```python
from build123d import *
from OCP.BRepFilletAPI import BRepFilletAPI_MakeChamfer

# Parameters (mm, degrees)
SKETCH_2_R              = 10.5
CUT_EXTRUDE_1_DEPTH     = 133.003787824
HOLE_WIZARD_M24_2_D     = 21
HOLE_WIZARD_M24_2_DEPTH = 63
HOLE_WIZARD_M24_2_TIP   = 6.3090365
CHAMFER_1_SIZE          = 2
CHAMFER_1_SIZE2         = 0.789861687


with BuildPart() as part:
    # 草图1 → 旋转1 (revolve)
    with BuildSketch(Plane.XY, mode=Mode.PRIVATE) as revolve_1_sk:
        Polygon((0, 0), (0, 26.473460386), (20, 30), (105, 30), (125, 26.473460386), (125, 0), align=None)
    revolve(revolve_1_sk.sketch.rotate(Axis((0, 0, 0), (1, 0, 0)), 90), axis=Axis((0, 0, 0), (1, 0, 0)))

    # 草图2 → 切除-拉伸1 (cut, through all)
    with BuildSketch(Plane(origin=(125, 0, 0), x_dir=(0, 0, -1), z_dir=(1, 0, 0))):
        Circle(SKETCH_2_R)
    extrude(amount=-CUT_EXTRUDE_1_DEPTH, mode=Mode.SUBTRACT)

    # M24 螺纹孔2
    with Locations(Plane(origin=(0, 0, 0), x_dir=(0, 0, -1), z_dir=(-1, 0, 0))):
        with Locations((0, 0)):
            Hole(HOLE_WIZARD_M24_2_D / 2, depth=HOLE_WIZARD_M24_2_DEPTH)
            with Locations((0, 0, -(HOLE_WIZARD_M24_2_DEPTH + HOLE_WIZARD_M24_2_TIP / 2))):  # 118° drill point
                Cone(0, HOLE_WIZARD_M24_2_D / 2, HOLE_WIZARD_M24_2_TIP, mode=Mode.SUBTRACT)

    # 倒角1: one chamfer whose edges measure the first distance from different faces: ONE call of the kernel's chamfer builder (chamfer() names one face for all edges)
    chamfer_1_edges_1 = [part.edges().sort_by_distance(p)[0] for p in [
        (0, 0, -26.473460386),
    ]]
    chamfer_1_side_1 = [part.faces().sort_by_distance(p)[0] for p in [
        (10, 0, -28.236730193),
    ]]
    chamfer_1_edges_2 = [part.edges().sort_by_distance(p)[0] for p in [
        (125, 0, -26.473460386),
    ]]
    chamfer_1_side_2 = [part.faces().sort_by_distance(p)[0] for p in [
        (115, 0, -28.236730193),
    ]]
    chamfer_1 = BRepFilletAPI_MakeChamfer(part.part.solid().wrapped)
    for e in chamfer_1_edges_1:
        chamfer_1.Add(CHAMFER_1_SIZE, CHAMFER_1_SIZE2, e.wrapped, chamfer_1_side_1[0].wrapped)  # the first distance lies on this face
    for e in chamfer_1_edges_2:
        chamfer_1.Add(CHAMFER_1_SIZE, CHAMFER_1_SIZE2, e.wrapped, chamfer_1_side_2[0].wrapped)  # the first distance lies on this face
    add(Compound.cast(chamfer_1.Shape()), mode=Mode.REPLACE)


solid = part.part
```
For this review, take the finished solid that the model builds, in its own axes (mm). Round coordinates to 2 decimals unless told otherwise and drop trailing zeros. Write each loop counter-clockwise with the first axis right and the second up, starting at its lowest first coordinate (ties: lowest second). Pieces come first, ordered by that corner, then holes. Notation, with made-up numbers: (2, 9) - (47, 9) arc R12 ccw to (47, 21) - close; hole circle Ø10 at (-34.75, 1.25). An arc over 180 degrees is marked (long way). Put each result on its own line as item: value.
Q1. Mouldability with a two-part tool opening along Y and no side actions: class faces 1 (the face through (0, 0, -11)), 2 (the face through (7.104, 27.067, -6.01)), 3 (the face through (63.4, 3.2, -10)) as released by +Y, released by -Y, zero draft, split by the parting line, or undercut.
Solved:
face 1: zero draft
face 2: split by the parting line
face 3: undercut
Q2. We need section D-D (x = 109.5). Give the boundary of the cut face in (y, z).
Solved:
outline: circle Ø58.41 at (0, 0); hole circle Ø21 at (0, 0)
Q3. We need section C-C (x = 44). Give the boundary of the cut face in (y, z).
Solved:
outline: circle Ø60 at (0, 0); hole circle Ø21 at (0, 0)
Q4. Insertion check: pin 1 Ø2 at (x, y) = (87.5, 6) entering from -Z; pin 2 Ø5 at (x, y) = (87, 9) entering from +Z; pin 3 Ø1 at (x, z) = (58, 1) entering from +Y. Each pin has a flat end and moves straight along its axis. Give the tip position at first contact, or say it passes through.
Solved:
pin 1: stops at z = -29.58
pin 2: stops at z = 29.29
pin 3: stops at y = 30
Q5. Wall thickness on probe 1 along Y at (x, z) = (73, 0); probe 2 along Z at (x, y) = (63, 5.5); probe 3 along Z at (x, y) = (107.5, -9.5): over which ranges is each line inside the solid? List them lowest first.
Solved:
probe 1: y = -30 to -10.5, 10.5 to 30
probe 2: z = -29.49 to -8.94, 8.94 to 29.49
probe 3: z = -27.99 to -4.47, 4.47 to 27.99
Q6. We need section A-A (z = 0). Give the boundary of the cut face in (x, y), and give its area (3 significant figures).
Solved:
outline: (0, -25.68) - (1.97, -26.82) - (20, -30) - (105, -30) - (123.03, -26.82) - (125, -25.68) - (125, -10.5) - (0, -10.5) - close; (0, 10.5) - (125, 10.5) - (125, 25.68) - (123.03, 26.82) - (105, 30) - (20, 30) - (1.97, 26.82) - (0, 25.68) - close
area: 4,730 mm2
